Could you check a few things on this model? Use its own coordinates, in mm. A direction names the side the tool comes from. Give positions to 0.01 mm unless a question says otherwise; leave off trailing zeros. Loops run counter-clockwise (first coordinate to the right, second up) from the corner with the lowest first, then second, coordinate; pieces in that order, holes last. Notation, with made-up numbers: M -34.75,-34.75 L 19.25,-34.75 A29 ccw 19.25,-7.75 Z; hole C 88.5,44 d11. An arc over 180 degrees is marked long. Answer in a Markdown table with one row per item. Add a question column.
1. If we section it at C-C on y = 29: List the corners of the cut face in (x, z) for me.
2. If we section it at A-A on x = 110: List the corners of the cut face in (y, z) for me, then the cut area to 3 significant figures.
3. Which directions (+Z, -Z, +X, -X, +Y, -Y) give clear straight access to the entire face, cutting with the end or side of a thin tool? Please do faces 1 (the flat face through (90, 33, 9)), 2 (the flat face through (15, 62, 35)), 3 (the flat face through (126.5, 26.1, 35)).
4. If we section it at B-B on x = 15: List the corners of the cut face in (y, z) for me, then the cut area to 3 significant figures.
5. Thinking about a two-plate mould opening in X: for faces 4 (the flat face through (150, 33, 0)), 5 (the flat face through (130, 33, 9)), 6 (the flat face through (0, 33, 9)), which applies, released by +X, released by -X, zero draft, split by the parting line, or undercut?
6. I'm going to push flat-ended pins straight in: pin 1 Ø6 at (x, y) = (50.5, 31.5) entering from +Z; pin 2 Ø1 at (x, y) = (110.5, 11.5) entering from -Z; pin 3 Ø5 at (y, z) = (38.5, 63.5) entering from +X; pin 4 Ø1.5 at (x, y) = (60, 44) entering from +Z. Where does each tip first touch, or does it pass through?
7. I need wall thicknesses on line 1 along Y through (x, z) = (110, 32.45); line 2 along Y through (x, z) = (110, 23); line 3 along Z through (x, y) = (15.5, 60.5). Which ranges of each line are inside material? Lowest first, please. Write a range as from..to.
8. If we section it at D-D on z = 52.5: List the corners of the cut face in (x, y) for me.
```python
from build123d import *

# Parameters (mm, degrees)
BASE_BLOCK_PROFILE_W    = 170
BASE_BLOCK_PROFILE_H    = 66
BASE_BLOCK_DEPTH        = 35
SLOT_CUT_DEPTH          = 66
COUNTERBORE_35_SKETCH_R = 17.5
COUNTERBORE_35_DEPTH    = 5
HOLE_20_SKETCH_R        = 10
HOLE_20_DEPTH           = 12
ROUNDED_CUT_DEPTH       = 30
SIDE_LUG_DEPTH          = 66
LUG_HOLE_16_SKETCH_R    = 8
LUG_HOLE_16_DEPTH       = 66


with BuildPart() as part:
    # Base Block Profile → Base Block (new body)
    with BuildSketch(Plane.XY):
        with Locations((85, 33)):
            Rectangle(BASE_BLOCK_PROFILE_W, BASE_BLOCK_PROFILE_H)
    extrude(amount=BASE_BLOCK_DEPTH)

    # Slot Profile → Slot Cut (cut)
    with BuildSketch(Plane.XZ):
        Polygon((110, 0), (130, 0), (130, 18), (90, 18), (90, 0), align=None)
    extrude(amount=-SLOT_CUT_DEPTH, mode=Mode.SUBTRACT)

    # Counterbore Ø35 Sketch → Counterbore Ø35 (cut)
    with BuildSketch(Plane.XY.offset(35)):
        with Locations((110, 33)):
            Circle(COUNTERBORE_35_SKETCH_R)
    extrude(amount=-COUNTERBORE_35_DEPTH, mode=Mode.SUBTRACT)

    # Hole Ø20 Sketch → Hole Ø20 (cut)
    with BuildSketch(Plane.XY.offset(30)):
        with Locations((110, 33)):
            Circle(HOLE_20_SKETCH_R)
    extrude(amount=-HOLE_20_DEPTH, mode=Mode.SUBTRACT)

    # Rounded Cut Sketch → Rounded Cut (cut)
    with BuildSketch(Plane.ZY):
        with BuildLine():
            Line((35, 58), (35, 8))
            ThreePointArc((35, 8), (10, 33), (35, 58))
        make_face()
    extrude(amount=-ROUNDED_CUT_DEPTH, mode=Mode.SUBTRACT)

    # Side Lug Profile → Side Lug (add)
    with BuildSketch(Plane.XZ):
        Polygon((30, 65), (30, 35), (60, 35), (60, 80), (50, 90), (0, 90), (0, 65), align=None)
    extrude(amount=-SIDE_LUG_DEPTH)

    # Lug Hole Ø16 Sketch → Lug Hole Ø16 (cut)
    with BuildSketch(Plane.XY.offset(90)):
        with Locations((15, 33)):
            Circle(LUG_HOLE_16_SKETCH_R)
    extrude(amount=-LUG_HOLE_16_DEPTH, mode=Mode.SUBTRACT)


solid = part.part
```
Results:
| question | item | result |
|---|---|---|
| 1 | outline | M 0,0 L 90,0 L 90,18 L 100.83,18 L 100.83,30 L 92.96,30 L 92.96,35 L 60,35 L 60,80 L 50,90 L 21.93,90 L 21.93,65 L 30,65 L 30,10.32 L 0,10.32 Z; M 0,65 L 8.07,65 L 8.07,90 L 0,90 Z; M 119.17,18 L 130,18 L 130,0 L 170,0 L 170,35 L 127.04,35 L 127.04,30 L 119.17,30 Z |
| 2 | outline | M 0,18 L 23,18 L 23,30 L 15.5,30 L 15.5,35 L 0,35 Z; M 43,18 L 66,18 L 66,35 L 50.5,35 L 50.5,30 L 43,30 Z |
| 2 | area | 707 mm2 |
| 3 | face 1 | -Z, +Y, -Y |
| 3 | face 2 | -X, +Y, -Y |
| 3 | face 3 | +Z, +X, +Y, -Y |
| 4 | outline | M 0,0 L 66,0 L 66,35 L 58,35 A25 cw 8,35 L 0,35 Z; M 0,65 L 25,65 L 25,90 L 0,90 Z; M 41,65 L 66,65 L 66,90 L 41,90 Z |
| 4 | area | 2,580 mm2 |
| 5 | face 4 | zero draft |
| 5 | face 5 | undercut |
| 5 | face 6 | released by -X |
| 6 | pin 1 | z = 90 |
| 6 | pin 2 | z = 18 |
| 6 | pin 3 | x = 60 |
| 6 | pin 4 | z = 80.75 |
| 7 | line 1 | 0..15.5, 50.5..66 |
| 7 | line 2 | 0..23, 43..66 |
| 7 | line 3 | 0..35, 65..90 |
| 8 | outline | M 30,0 L 60,0 L 60,66 L 30,66 Z |
